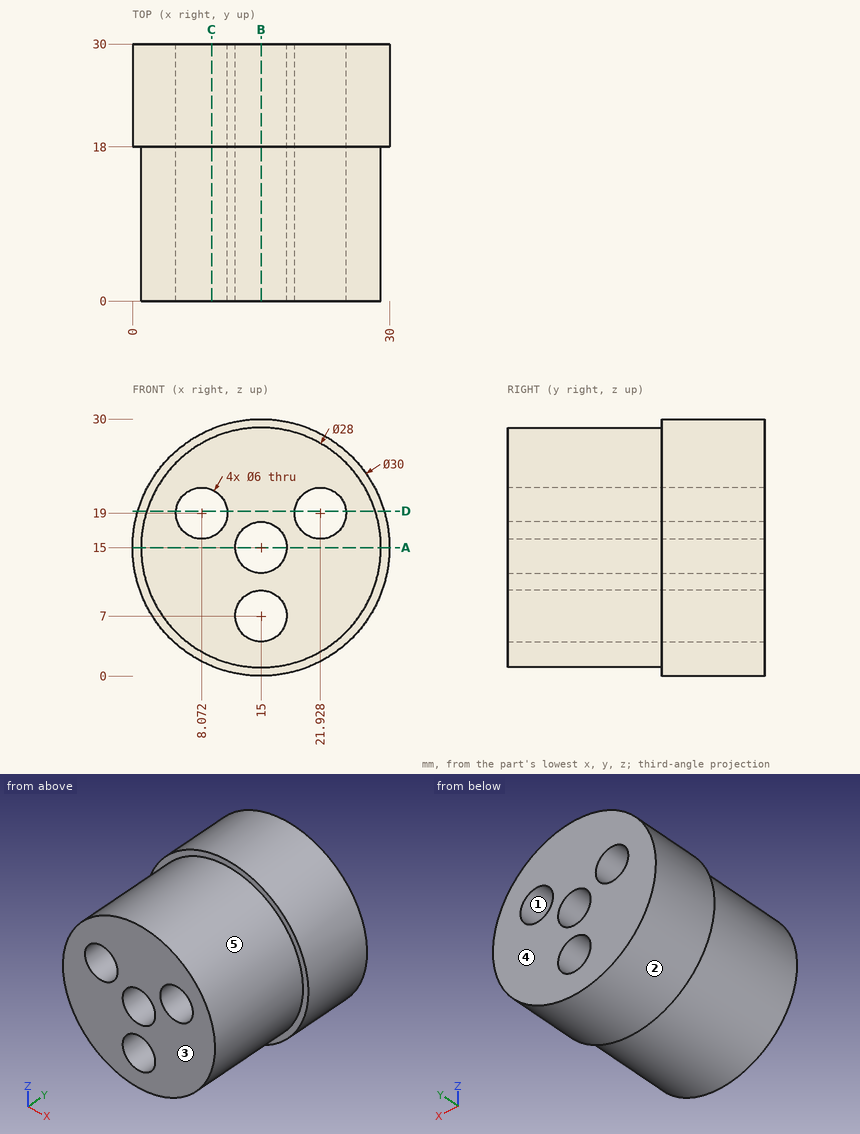
Here's the drawing with two shaded views (mm, measured from the low corner). I have some questions. A direction names the side the tool comes from. Coordinates: 2 decimals unless noted, no trailing zeros. Write each loop counter-clockwise with the first axis right and the second up, starting at its lowest first coordinate (ties: lowest second). Pieces come first, ordered by that corner, then holes. Notation, with made-up numbers: (-12.5, 55.25) -> (30.5, 55.25) arc R18 cw to (30.5, 73.25) -> close; hole circle Ø9 at (67, 32.25). An arc over 180 degrees is marked (long way). One line per question, with ' | ' between items. Start each with the question number.
1. If we section it at C-C (x = 9.25): Please give me the cut outline in (y, z) (1 decimal).
2. If we section it at A-A (z = 15): Please give me the cut outline in (x, y).
3. Thinking about a two-plate mould opening in Z: for the marked faces 1, 2 and 3, which applies, pulls with the +Z half, pulls with the -Z half, needs draft (parallel to the pull), parting line crosses it, or undercut?
4. If we section it at B-B (x = 15): Please give me the cut outline in (y, z).
5. If we section it at D-D (z = 19.25): Please give me the cut outline in (x, y) (1 decimal), and give its area (3 significant figures).
6. Will these pins go through, and if not, where does the flat tip stop? P1, Ø6, axis at x = 6.5, y = 15, coming from the -Z side; P2, Ø1.5, axis at x = 26.5, y = 17, coming from the -Z side; P3, Ø1, axis at y = 12.5, z = 11, coming from the -X side.
7. For the marked faces 4 and 5, which set-ups out of +Z, -Z, +X, -X, +Y, -Y let a thin tool reach every point of the face, with its end or its side?
8. Please list where these lines run through material, in increasing order: line 1 along X through (y, z) = (22.75, 19); line 2 along Z through (x, y) = (16.25, 25.75); line 3 along X through (y, z) = (15.25, 19).
Return value:
1) outline: (0, 2.2) -> (18, 2.2) -> (18, 1.1) -> (30, 1.1) -> (30, 16.2) -> (0, 16.2) -> close; (0, 21.8) -> (30, 21.8) -> (30, 28.9) -> (18, 28.9) -> (18, 27.8) -> (0, 27.8) -> close
2) outline: (0, 18) -> (1, 18) -> (1, 0) -> (12, 0) -> (12, 30) -> (0, 30) -> close; (18, 0) -> (29, 0) -> (29, 18) -> (30, 18) -> (30, 30) -> (18, 30) -> close
3) face 1: undercut | face 2: parting line crosses it | face 3: needs draft
4) outline: (0, 1) -> (18, 1) -> (18, 0) -> (30, 0) -> (30, 4) -> (0, 4) -> close; (0, 10) -> (30, 10) -> (30, 12) -> (0, 12) -> close; (0, 18) -> (30, 18) -> (30, 30) -> (18, 30) -> (18, 29) -> (0, 29) -> close
5) outline: (0.6, 18) -> (1.7, 18) -> (1.7, 0) -> (5.1, 0) -> (5.1, 30) -> (0.6, 30) -> close; (11.1, 0) -> (18.9, 0) -> (18.9, 30) -> (11.1, 30) -> close; (24.9, 0) -> (28.3, 0) -> (28.3, 18) -> (29.4, 18) -> (29.4, 30) -> (24.9, 30) -> close | area: 467 mm²
6) P1: stops at z = 2.13 | P2: stops at z = 6.03 | P3: stops at x = 1.44
7) face 4: +Z, -Z, +X, -X, +Y | face 5: -Y
8) line 1: x = 0.54 to 5.07, 11.07 to 18.93, 24.93 to 29.46 | line 2: z = 0.05 to 4.27, 9.73 to 12.27, 17.73 to 29.95 | line 3: x = 1.58 to 5.07, 11.07 to 18.93, 24.93 to 28.42
